```python
from build123d import *

# Parameters (mm, degrees)
HOLE_WIZARD_M6_1_D        = 5
HOLE_WIZARD_M6_1_DEPTH    = 17
HOLE_WIZARD_M6_1_TIP      = 1.502151548
CHAMFER_1_SIZE            = 0.5
HOLE_WIZARD_6_0_6_1_D     = 6
HOLE_WIZARD_6_0_6_1_DEPTH = 10
HOLE_WIZARD_6_0_6_1_TIP   = 1.802581857


with BuildPart() as part:
    # 草图1 → 旋转1 (revolve)
    with BuildSketch(Plane.XY, mode=Mode.PRIVATE) as revolve_1_sk:
        Polygon((4.5, 10), (0, 10), (0, 0), (74, 0), (74, 20), (64.5, 20), (40.5, 10.058874503), (40.5, 10), (34.5, 10), (31.820508076, 20), (28.5, 20), (4.5, 10.058874503), align=None)
    revolve(revolve_1_sk.sketch.rotate(Axis((0, 0, 0), (1, 0, 0)), 90), axis=Axis((0, 0, 0), (1, 0, 0)))

    # M6 螺纹孔1
    with Locations(Plane(origin=(74, 0, 0), x_dir=(0, 0, -1), z_dir=(1, 0, 0))):
        with Locations((0, 0)):
            Hole(HOLE_WIZARD_M6_1_D / 2, depth=HOLE_WIZARD_M6_1_DEPTH)
            with Locations((0, 0, -(HOLE_WIZARD_M6_1_DEPTH + HOLE_WIZARD_M6_1_TIP / 2))):  # 118° drill point
                Cone(0, HOLE_WIZARD_M6_1_D / 2, HOLE_WIZARD_M6_1_TIP, mode=Mode.SUBTRACT)

    # 倒角1
    chamfer_1_edges = [part.edges().sort_by_distance(p)[0] for p in [
        (74, 0, -2.5),
    ]]
    chamfer(chamfer_1_edges, length=CHAMFER_1_SIZE)

    # Ø6.0 (6) 直径孔1
    with Locations(Plane(origin=(69, 0, 20), x_dir=(1, 0, 0), z_dir=(0, 0, 1))):
        with Locations((0, 0)):
            Hole(HOLE_WIZARD_6_0_6_1_D / 2, depth=HOLE_WIZARD_6_0_6_1_DEPTH)
            with Locations((0, 0, -(HOLE_WIZARD_6_0_6_1_DEPTH + HOLE_WIZARD_6_0_6_1_TIP / 2))):  # 118° drill point
                Cone(0, HOLE_WIZARD_6_0_6_1_D / 2, HOLE_WIZARD_6_0_6_1_TIP, mode=Mode.SUBTRACT)


solid = part.part
```
For this review, take the finished solid that the model builds, in its own axes (mm). A direction names the side the tool comes from. Round coordinates to 2 decimals unless told otherwise and drop trailing zeros. Write each loop counter-clockwise with the first axis right and the second up, starting at its lowest first coordinate (ties: lowest second). Pieces come first, ordered by that corner, then holes. Notation, with made-up numbers: M -21,15 L 35,15 A13 ccw 35,19 Z; hole C 0,26.5 d10. An arc over 180 degrees is marked long. One line per item, written item: value. Start each with the question number.
(1) Machinability: for faces 4 (the cylindrical face through (37, 0, -10)), 5 (the cylindrical face through (2, 0, -10)), 6 (the cylindrical face through (71.4, -1.8, 14.9)), which of the approach directions +Z, -Z, +X, -X, +Y, -Y give a long, thin tool a straight path to every point of the face, cutting with its end or side? Answer none if there is none.
(2) We need section A-A (x = 19). Give the boundary of the cut face in (y, z).
(3) We need section B-B (x = 52). Give the boundary of the cut face in (y, z).
(4) The part is to be moulded in two halves that separate along Z. For faces 1 (the cylindrical face through (69.18, -0.88, -19.98)), 2 (the conical face through (68.62, 0.35, 8.51)), 3 (the cylindrical face through (65.13, -2.44, -0.54)), say which applies: released by +Z, released by -Z, zero draft, split by the parting line, or undercut.
(5) Wall thickness on line 1 (X direction, y = -1, z = 10); line 2 (Z direction, x = 70, y = 0); line 3 (X direction, y = -11.5, z = 9): over which ranges is each line inside the solid? List them lowest first.
(6) Insertion check: pin 1 (2 mm diameter, centred on x = 48.5, z = -14.5, fed in from -Y); pin 2 (12 mm diameter, centred on y = -2.5, z = -7.5, fed in from -X); pin 3 (1 mm diameter, centred on x = 30.5, y = 9, fed in from -Z); pin 4 (1 mm diameter, centred on x = 28, z = -6, fed in from -Y). Each pin has a flat end and moves straight along its axis. Give the tip position at first contact, or say it passes through.
Result:
1. face 4: none
1. face 5: -X
1. face 6: +Z
2. outline: C 0,0 d32.13
3. outline: C 0,0 d29.64
4. face 1: split by the parting line
4. face 2: released by +Z
4. face 3: undercut
5. line 1: 4.5 to 34.49, 40.5 to 66.17, 71.83 to 74
5. line 2: -20 to -2.5, 2.5 to 8.8
5. line 3: 15.47 to 33.27, 51.47 to 74
6. pin 1: through
6. pin 2: x = 0
6. pin 3: z = -18.1
6. pin 4: y = -19.13
